from build123d import *

# Parameters (mm, degrees)
SKETCH_1_W          = 325
SKETCH_1_H          = 240
EXTRUDE_1_DEPTH     = 40
SKETCH_2_W          = 185
SKETCH_2_H          = 185
CUT_EXTRUDE_1_DEPTH = 23
SKETCH_3_R          = 70
CUT_EXTRUDE_2_DEPTH = 204.310722787
FILLET_1_R          = 5
CHAMFER_1_SIZE      = 15


with BuildPart() as part:
    # 草图1 → 凸台-拉伸1 (new body)
    with BuildSketch(Plane(origin=(0, 0, 0), x_dir=(1, 0, 0), z_dir=(0, 1, 0))):
        Rectangle(SKETCH_1_W, SKETCH_1_H)
    extrude(amount=EXTRUDE_1_DEPTH)

    # 草图2 → 切除-拉伸1 (cut)
    with BuildSketch(Plane.XZ):
        with Locations((-51.793832524, 0)):
            Rectangle(SKETCH_2_W, SKETCH_2_H)
    extrude(amount=-CUT_EXTRUDE_1_DEPTH, mode=Mode.SUBTRACT)

    # 草图3 → 切除-拉伸2 (cut, through all)
    with BuildSketch(Plane.XZ.offset(-23)):
        with Locations(Location((-51.793832524, 0, 0), (0, 0, 270))):
            Circle(SKETCH_3_R)
    extrude(amount=-CUT_EXTRUDE_2_DEPTH, mode=Mode.SUBTRACT)

    # 圆角1
    fillet_1_edges = [part.edges().sort_by_distance(p)[0] for p in [
        (-144.293832524, 11.5, -92.5),
        (-144.293832524, 11.5, 92.5),
        (40.706167476, 11.5, 92.5),
        (40.706167476, 11.5, -92.5),
    ]]
    fillet(fillet_1_edges, radius=FILLET_1_R)

    # 倒角1
    chamfer_1_edges = [part.edges().sort_by_distance(p)[0] for p in [
        (162.5, 20, 120),
        (162.5, 20, -120),
    ]]
    chamfer(chamfer_1_edges, length=CHAMFER_1_SIZE)


solid = part.part
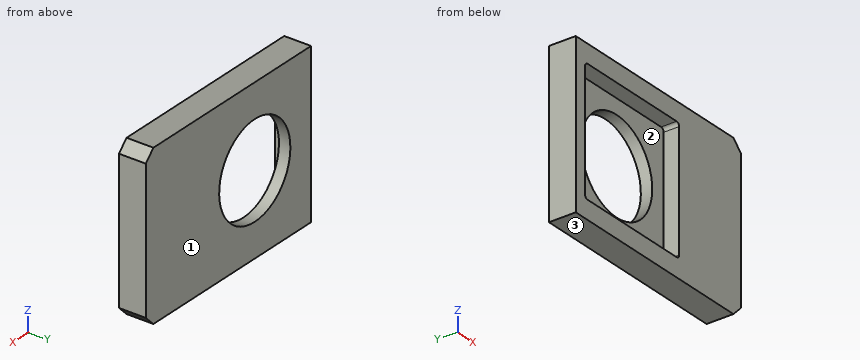
Read the model definition and answer for the solid it produces. Units are mm, in the model's axes. Face numbers are marked on the shaded views. Coordinates: 2 decimals unless noted, no trailing zeros. Order: outer loops, then holes, each group sorted by start corner. A loop starts at its lowest first (then second) coordinate and runs counter-clockwise, first axis right, second up. Notation, with made-up numbers: (-8.5, -19.5) - (43.5, -19.5) arc R22 ccw to (43.5, 7.5) - close; hole circle Ø8 at (25, -34.75). An arc over 180 degrees is marked (long way). Use one line per item in the form item = value.
(1) Section D-D, the plane x = -132 is taken. Give the vertices of the cut face in (y, z), then the cut area to 4 significant figures.
Computed values:
outline = (0, -120) - (40, -120) - (40, 120) - (0, 120) - (0, 92.5) - (23, 92.5) - (23, -92.5) - (0, -92.5) - close
area = 5,345 mm²
(2) Section A-A, the plane z = 0 is taken. Give the vertices of the cut face in (x, y).
Computed values:
outline = (-162.5, 0) - (-144.29, 0) - (-144.29, 23) - (-121.79, 23) - (-121.79, 40) - (-162.5, 40) - close; (18.21, 23) - (40.71, 23) - (40.71, 0) - (162.5, 0) - (162.5, 40) - (18.21, 40) - close
(3) For a pull along Z with two mould halves and no side action, classify the marked faces 1, 2 and 3 as pulls with the +Z half, pulls with the -Z half, needs draft (parallel to the pull), parting line crosses it, or undercut.
Computed values:
face_1 = needs draft
face_2 = undercut
face_3 = pulls with the -Z half
(4) Straight lines are drawn through the part: L1, parallel to X at y = 29.5, z = 0; L2, parallel to X at y = 15.5, z = -69.5; L3, parallel to Z at x = -47.5, y = 21. For each, find the intervals that lie inside material, in ascending order.
Computed values:
L1 = -162.5 to -121.79, 18.21 to 162.5
L2 = -162.5 to -144.29, 40.71 to 162.5
L3 = -120 to -92.5, 92.5 to 120
(5) Section B-B, the plane y = 4 is taken. Give the vertices of the cut face in (x, z), then the cut area to 3 significant figures.
Computed values:
outline = (-162.5, -120) - (147.5, -120) - (162.5, -105) - (162.5, 105) - (147.5, 120) - (-162.5, 120) - close; hole (-144.29, -87.5) arc R5 ccw to (-139.29, -92.5) - (35.71, -92.5) arc R5 ccw to (40.71, -87.5) - (40.71, 87.5) arc R5 ccw to (35.71, 92.5) - (-139.29, 92.5) arc R5 ccw to (-144.29, 87.5) - close
area = 43,600 mm²
(6) Section C-C, the plane x = -41 is taken. Give the vertices of the cut face in (y, z).
Computed values:
outline = (0, -120) - (40, -120) - (40, -69.16) - (23, -69.16) - (23, -92.5) - (0, -92.5) - close; (0, 92.5) - (23, 92.5) - (23, 69.16) - (40, 69.16) - (40, 120) - (0, 120) - close
